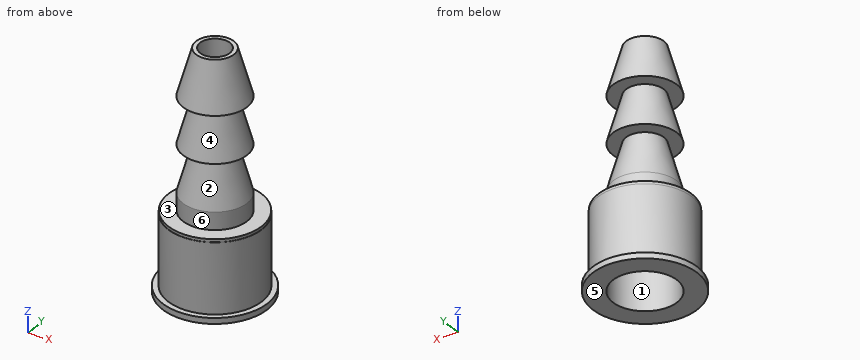
from build123d import *

# Parameters (mm, degrees)
FLANGE_SKETCH_R        = 9
FLANGE_DEPTH           = 1
BODY_SKETCH_R          = 8.05
BODY_DEPTH             = 12
SHOULDER_STEP_SKETCH_R = 8
SHOULDER_STEP_DEPTH    = 0.5
NECK_SKETCH_R          = 5.5
NECK_DEPTH             = 3
BARB_1_SKETCH_R        = 5.5
BARB_1_DEPTH           = 8
BARB_1_TAPER           = 15.66
BARB_2_SKETCH_R        = 5.5
BARB_2_DEPTH           = 8
BARB_2_TAPER           = 15.66
BARB_3_SKETCH_R        = 5.5
BARB_3_TIP_DEPTH       = 8
BARB_3_TIP_TAPER       = 15.66
INLET_BORE_SKETCH_R    = 5.5
INLET_BORE_DEPTH       = 12
THROUGH_BORE_SKETCH_R  = 2.55
THROUGH_BORE_DEPTH     = 38


with BuildPart() as part:
    # Flange Sketch → Flange (new body)
    with BuildSketch(Plane.XY):
        Circle(FLANGE_SKETCH_R)
    extrude(amount=FLANGE_DEPTH)

    # Body Sketch → Body (add)
    with BuildSketch(Plane.XY.offset(1)):
        Circle(BODY_SKETCH_R)
    extrude(amount=BODY_DEPTH)

    # Shoulder Step Sketch → Shoulder Step (add)
    with BuildSketch(Plane.XY.offset(13)):
        Circle(SHOULDER_STEP_SKETCH_R)
    extrude(amount=SHOULDER_STEP_DEPTH)

    # Neck Sketch → Neck (add)
    with BuildSketch(Plane.XY.offset(13.5)):
        Circle(NECK_SKETCH_R)
    extrude(amount=NECK_DEPTH)

    # Barb 1 Sketch → Barb 1 (add)
    with BuildSketch(Plane.XY.offset(16.5)):
        Circle(BARB_1_SKETCH_R)
    extrude(amount=BARB_1_DEPTH, taper=BARB_1_TAPER)

    # Barb 2 Sketch → Barb 2 (add)
    with BuildSketch(Plane.XY.offset(24.5)):
        Circle(BARB_2_SKETCH_R)
    extrude(amount=BARB_2_DEPTH, taper=BARB_2_TAPER)

    # Barb 3 Sketch → Barb 3 Tip (add)
    with BuildSketch(Plane.XY.offset(32.5)):
        Circle(BARB_3_SKETCH_R)
    extrude(amount=BARB_3_TIP_DEPTH, taper=BARB_3_TIP_TAPER)

    # Inlet Bore Sketch → Inlet Bore (cut)
    with BuildSketch(Plane(origin=(0, 0, 0), x_dir=(-1, 0, 0), z_dir=(0, 0, -1))):
        with Locations(Location((0, 0, 0), (0, 0, 180))):
            Circle(INLET_BORE_SKETCH_R)
    extrude(amount=-INLET_BORE_DEPTH, mode=Mode.SUBTRACT)

    # Through Bore Sketch → Through Bore (cut)
    with BuildSketch(Plane(origin=(0, 0, 12), x_dir=(-1, 0, 0), z_dir=(0, 0, -1))):
        Circle(THROUGH_BORE_SKETCH_R)
    extrude(amount=-THROUGH_BORE_DEPTH, mode=Mode.SUBTRACT)


solid = part.part
Part model, mm, in its own coordinate system. Face numbers are marked on the shaded views. A direction names the side the tool comes from. Give positions to 0.01 mm unless a question says otherwise; leave off trailing zeros. Order: outer loops, then holes, each group sorted by start corner. A loop starts at its lowest first (then second) coordinate and runs counter-clockwise, first axis right, second up. Notation, with made-up numbers: (85, 41) - (141, 41) arc R32 cw to (141, 76) - close; hole circle Ø9 at (-29, -38.75). An arc over 180 degrees is marked (long way). Use a Markdown table: item, result.
1) Two-plate mould, pull along Z, no slides. Class the marked faces 4, 5 and 6: +Z half, -Z half, draft (parallel to the pull), parting line (faces both ways), or undercut.
Checked values:
| item | result |
|---|---|
| face 4 | undercut |
| face 5 | -Z half |
| face 6 | draft |
2) Probe L1, parallel to Y at x = 0, z = 8.75; L2, parallel to Y at x = 0.5, z = 34; L3, parallel to X at y = -1.5, z = 19. List the from-to ranges inside material, lowest first. Write a range as from..to.
Checked values:
| item | result |
|---|---|
| L1 | -8.05..-5.5, 5.5..8.05 |
| L2 | -5.05..-2.5, 2.5..5.05 |
| L3 | -4.56..-2.06, 2.06..4.56 |
3) Saw through at D-D on x = -4.25. Count the separate pieces of the cut face and the enclosed holes in it, plus the area to 3 significant figures.
Checked values:
| item | result |
|---|---|
| separate pieces | 3 |
| enclosed holes | 0 |
| area | 185 mm² |
4) 3-axis set-ups, long thin cutter, end or side, ignore diameter. For the marked faces 1, 2 and 3: which of +Z, -Z, +X, -X, +Y, -Y reach the whole face in a straight line?
Checked values:
| item | result |
|---|---|
| face 1 | -Z |
| face 2 | none |
| face 3 | +Z |
5) Flat gauge pins, fed straight in: P1, Ø1.5, axis at x = 6.5, z = 36, coming from the -Y side; P2, Ø5.5, axis at x = 0.5, y = 1.5, coming from the -Z side; P3, Ø8, axis at x = -0.5, z = 19, coming from the +Y side; P4, Ø8, axis at x = 2, z = 6.5, coming from the -Y side. Where does each tip first touch, or does it go through?
Checked values:
| item | result |
|---|---|
| P1 | through |
| P2 | z = 12 |
| P3 | y = 5.5 |
| P4 | y = -8.05 |
6) Saw through at C-C on z = 33.5. List the corners of the cut face in (x, y), plus the area to 3 significant figures.
Checked values:
| item | result |
|---|---|
| outline | circle Ø10.44 at (0, 0); hole circle Ø5.1 at (0, 0) |
| area | 65.2 mm² |
